Geometry check sheet. Reference: the model listing, model coordinates, mm. A direction names the side the tool comes from. Coordinates: 2 decimals unless noted, no trailing zeros. Order: outer loops, then holes, each group sorted by start corner. A loop starts at its lowest first (then second) coordinate and runs counter-clockwise, first axis right, second up.
```python
from build123d import *

# Parameters (mm, degrees)
SKETCH1_R = 22.5
SHELL1_T  = -2


with BuildPart() as part:
    # Sweep1: sweep along a path in Sketch2
    with BuildLine(Plane(origin=(0, 0, 0), x_dir=(1, 0, 0), z_dir=(0, 1, 0))) as sweep1_path:
        Line((0, 0), (0, 29.998925194))
        ThreePointArc((0, 29.998925194), (5.808917204, 56.201257422), (22.147168199, 77.493680668))
        Line((22.147168199, 77.493680668), (62.502026728, 111.355427576))
    # Sketch1 → Sweep1 (sweep)
    with BuildSketch(Plane.XY):
        Circle(SKETCH1_R)
    sweep(path=sweep1_path.line)

    # Shell1
    shell1_openings = [part.faces().sort_by_distance(p)[0] for p in [
        (62.502026728, 0, -111.355427576),
        (0, 0, 0),
    ]]
    offset(amount=SHELL1_T, openings=shell1_openings, kind=Kind.INTERSECTION)


solid = part.part
```
Item 1: Sectioned sample at A-A (y = -19). Record the cut outline in (x, z), and give its area (3 significant figures).
Item 2: Sectioned sample at C-C (y = 0). Record the cut outline in (x, z).
Item 3: Thickness scan on line 1 along X through (y, z) = (0, -21); line 2 along Y through (x, z) = (51.5, -120). Record the ranges inside material, lowest first.
Item 4: Release check for a two-part mould opening along Y. For faces 3 (the face through (-4.444, 20.013, -15.209)), 4 (the face through (55.176, -6.158, -79.683)), 5 (the face through (56.14, 18.23, -118.94)), 6 (the face through (55.967, 8.618, -78.74)) record: pulls with the +Y half, pulls with the -Y half, needs draft (parallel to the pull), parting line crosses it, or undercut.
Item 5: Sectioned sample at B-B (z = -25.5). Record the cut outline in (x, y), and give its area (3 significant figures).
Item 6: Tool access check on faces 1 (the face through (10.382, 19.961, -15.209)), 2 (the face through (9.9, -18.2, 0)). Record the directions out of +Z, -Z, +X, -X, +Y, -Y that give a thin tool (end or side, any length) a straight path to the whole face; none if there is none.
Item 7: Depth check by flat-ended pin: P1, Ø6, axis at x = 62, z = -91, coming from the +Y side; P2, Ø10, axis at y = -5, z = -80, coming from the +X side; P3, Ø10, axis at y = -8, z = -34, coming from the -X side. Enter the tip coordinate at first touch or a pass-through.
Geometry check:
1. outline: (-12.05, -30) arc R74.05 ccw to (14.4, -86.73) - (54.76, -120.59) - (57.55, -117.25) - (17.2, -83.39) arc R69.7 cw to (-7.7, -30) - (-7.7, 0) - (-12.05, 0) - close; (7.7, -30) arc R54.3 ccw to (27.09, -71.6) - (67.45, -105.46) - (70.25, -102.12) - (29.89, -68.26) arc R49.95 cw to (12.05, -30) - (12.05, 0) - (7.7, 0) - close
1. area: 1,190 mm2
2. outline: (-22.5, -30) arc R84.5 ccw to (7.68, -94.73) - (48.04, -128.59) - (49.32, -127.06) - (8.97, -93.2) arc R82.5 cw to (-20.5, -30) - (-20.5, 0) - (-22.5, 0) - close; (20.5, -30) arc R41.5 ccw to (35.32, -61.79) - (75.68, -95.65) - (76.96, -94.12) - (36.61, -60.26) arc R39.5 cw to (22.5, -30) - (22.5, 0) - (20.5, 0) - close
3. line 1: x = -22.5 to -20.5, 20.5 to 22.5
3. line 2: y = -17.85 to -15.26, 15.26 to 17.85
4. face 3: undercut
4. face 4: undercut
4. face 5: needs draft
4. face 6: parting line crosses it
5. outline: circle Ø45 at (0, 0); hole circle Ø41 at (0, 0)
5. area: 270 mm2
6. face 1: +Z
6. face 2: +Z, +X, -X, +Y, -Y
7. P1: stops at y = 18.86
7. P2: stops at x = 65.42
7. P3: stops at x = -22.23
